Verification items for the finished model (mm, model axes). A direction names the side the tool comes from. Give positions to 0.01 mm unless a question says otherwise; leave off trailing zeros. Order: outer loops, then holes, each group sorted by start corner. A loop starts at its lowest first (then second) coordinate and runs counter-clockwise, first axis right, second up. Notation, with made-up numbers: (19, 50.5) - (38, 50.5) arc R16 ccw to (38, 77.5) - close; hole circle Ø5 at (-1.5, 85.5). An arc over 180 degrees is marked (long way). Answer as a JSON object with one key per item and string values.
```python
from build123d import *

# Parameters (mm, degrees)
SKETCH_1_W                = 140
SKETCH_1_H                = 55
EXTRUDE_1_DEPTH           = 12
SKETCH_2_W                = 10.2
SKETCH_2_H                = 67.741828953
CUT_EXTRUDE_1_DEPTH       = 2
CHAMFER_1_SIZE            = 1
CUT_EXTRUDE_2_DEPTH       = 36
HOLE_WIZARD_0_D           = 4.4
HOLE_WIZARD_0_CBORE_D     = 8
HOLE_WIZARD_0_CBORE_DEPTH = 5


with BuildPart() as part:
    # 草图1 → 凸台-拉伸1 (new body)
    with BuildSketch(Plane(origin=(0, 0, 0), x_dir=(0, 0, -1), z_dir=(1, 0, 0))):
        Rectangle(SKETCH_1_W, SKETCH_1_H)
    extrude(amount=EXTRUDE_1_DEPTH)

    # 草图2 → 切除-拉伸1 (cut)
    with BuildSketch(Plane(origin=(12, 0, 0), x_dir=(0, 0, -1), z_dir=(1, 0, 0))):
        with Locations((-61, -0.529795054)):
            Rectangle(SKETCH_2_W, SKETCH_2_H)
    cut_extrude_1 = extrude(amount=-CUT_EXTRUDE_1_DEPTH, mode=Mode.SUBTRACT)

    # 倒角1
    chamfer_1_edges = [part.edges().sort_by_distance(p)[0] for p in [
        (6, -27.5, -70),
        (6, 27.5, -70),
    ]]
    chamfer(chamfer_1_edges, length=CHAMFER_1_SIZE)

    # 镜向2: 切除-拉伸1 across plane
    add(cut_extrude_1.mirror(Plane.XY), mode=Mode.SUBTRACT)

    # 草图3 → 切除-拉伸2 (cut)
    with BuildSketch(Plane(origin=(12, 0, 0), x_dir=(0, 0, -1), z_dir=(1, 0, 0))):
        with BuildLine():
            Line((-45, 23.25), (-25, 23.25))
            ThreePointArc((-25, 23.25), (-21.75, 20), (-25, 16.75))
            Line((-25, 16.75), (-45, 16.75))
            ThreePointArc((-45, 16.75), (-48.25, 20), (-45, 23.25))
        make_face()
        with BuildLine():
            Line((-45, -23.25), (-25, -23.25))
            ThreePointArc((-25, -23.25), (-21.75, -20), (-25, -16.75))
            Line((-25, -16.75), (-45, -16.75))
            ThreePointArc((-45, -16.75), (-48.25, -20), (-45, -23.25))
        make_face()
        with BuildLine():
            Line((45, 23.25), (25, 23.25))
            ThreePointArc((25, 23.25), (21.75, 20), (25, 16.75))
            Line((25, 16.75), (45, 16.75))
            ThreePointArc((45, 16.75), (48.25, 20), (45, 23.25))
        make_face()
        with BuildLine():
            Line((45, -23.25), (25, -23.25))
            ThreePointArc((25, -23.25), (21.75, -20), (25, -16.75))
            Line((25, -16.75), (45, -16.75))
            ThreePointArc((45, -16.75), (48.25, -20), (45, -23.25))
        make_face()
    extrude(amount=-CUT_EXTRUDE_2_DEPTH, mode=Mode.SUBTRACT)

    # 打孔尺寸(%根据)内六角圆柱头螺钉的类型0 (through all)
    with Locations(Plane.ZY):
        with Locations((-61, 18), (-61, -18), (61, 18), (61, -18)):
            CounterBoreHole(HOLE_WIZARD_0_D / 2, HOLE_WIZARD_0_CBORE_D / 2, HOLE_WIZARD_0_CBORE_DEPTH)


solid = part.part
```
(1) Section check A-A (z = 61). Record the cut outline in (x, y).
Computed values:
{"outline": "(0, -27.5) - (10, -27.5) - (10, -20.2) - (5, -20.2) - (5, -22) - (0, -22) - close; (0, -14) - (5, -14) - (5, -15.8) - (10, -15.8) - (10, 15.8) - (5, 15.8) - (5, 14) - (0, 14) - close; (0, 22) - (5, 22) - (5, 20.2) - (10, 20.2) - (10, 27.5) - (0, 27.5) - close"}
(2) Gauge pin test, flat ends, axial feed: pin 1 Ø8 at (y, z) = (-12.5, 62) entering from +X; pin 2 Ø7 at (y, z) = (18, 61) entering from -X. Record the tip position at first contact, or that the pin passes through.
Computed values:
{"pin 1": "stops at x = 10", "pin 2": "stops at x = 5"}
(3) Material ranges on line 1 along Y through (x, z) = (1.1, 61); line 2 along Y through (x, z) = (7.45, 61); line 3 along Z through (x, y) = (8.25, -16), recorded low to high. Write a range as [from, to].
Computed values:
{"line 1": "y = [-27.5, -22], [-14, 14], [22, 27.5]", "line 2": "y = [-27.5, -20.2], [-15.8, 15.8], [20.2, 27.5]", "line 3": "z = [-70, -61.92], [-60.08, 60.08], [61.92, 70]"}
(4) Section check B-B (y = 1.5). Record the cut outline in (x, z).
Computed values:
{"outline": "(0, -70) - (12, -70) - (12, -66.1) - (10, -66.1) - (10, -55.9) - (12, -55.9) - (12, 55.9) - (10, 55.9) - (10, 66.1) - (12, 66.1) - (12, 70) - (0, 70) - close"}
(5) Section check C-C (z = -38). Record the cut outline in (x, y), then the cut area to 3 significant figures.
Computed values:
{"outline": "(0, -27.5) - (12, -27.5) - (12, -23.25) - (0, -23.25) - close; (0, -16.75) - (12, -16.75) - (12, 16.75) - (0, 16.75) - close; (0, 23.25) - (12, 23.25) - (12, 27.5) - (0, 27.5) - close", "area": "504 mm²"}
(6) Section check D-D (y = 18). Count the separate pieces of the cut face and the enclosed holes in it, then the cut area to 3 significant figures.
Computed values:
{"separate pieces": "5", "enclosed holes": "0", "area": "912 mm²"}
(7) Release check for a two-part mould opening along Z. For faces 4 (the flat face through (12, 0, 68)), 5 (the flat face through (6, 0, -70)), 6 (the cylindrical face through (6.08, 19.93, 48.25)) record: pulls with the +Z half, pulls with the -Z half, needs draft (parallel to the pull), parting line crosses it, or undercut.
Computed values:
{"face 4": "needs draft", "face 5": "pulls with the -Z half", "face 6": "undercut"}
(8) Access from +Z, -Z, +X, -X, +Y, -Y to the whole of each face (thin tool, end or side, straight path). Record for faces 1 (the flat face through (5, 16, -59)), 2 (the flat face through (6, 16.75, -35)), 3 (the flat face through (6, -27.5, 1)).
Computed values:
{"face 1": "-X", "face 2": "+X, -X", "face 3": "+Z, -Z, +X, -X, -Y"}
